from build123d import *

# Parameters (mm, degrees)
SKETCH1_R           = 36.5
BOSS_EXTRUDE1_DEPTH = 268
SKETCH2_R           = 70
SKETCH2_R_2         = 55
CUT_EXTRUDE1_DEPTH  = 36
CUT_EXTRUDE2_START  = -36
SKETCH3_R           = 70
SKETCH3_R_2         = 55
CUT_EXTRUDE2_DEPTH  = 36


with BuildPart() as part:
    # Sketch1 → Boss-Extrude1 (new body)
    with BuildSketch(Plane.XY):
        with BuildLine():
            Line((-40.165283517, 53), (-10.3, 53))
            Line((-10.3, 53), (-10.3, 65.697488536))
            ThreePointArc((-10.3, 65.697488536), (66.373170096, 4.105154246), (-2.125739686, -66.466015608))
            Line((-2.125739686, -66.466015608), (-4.128100838, -53.823604848))
            Line((-4.128100838, -53.823604848), (-32.079680877, -58.250700209))
            ThreePointArc((-32.079680877, -58.250700209), (-66.325057816, -4.820446627), (-40.165283517, 53))
        make_face()
        Circle(SKETCH1_R, mode=Mode.SUBTRACT)
    extrude(amount=BOSS_EXTRUDE1_DEPTH)

    # Sketch2 → Cut-Extrude1 (cut)
    with BuildSketch(Plane.XY.offset(268)):
        Circle(SKETCH2_R)
        Circle(SKETCH2_R_2, mode=Mode.SUBTRACT)
    extrude(amount=-CUT_EXTRUDE1_DEPTH, mode=Mode.SUBTRACT)

    # Sketch3 → Cut-Extrude2 (cut)
    with BuildSketch(Plane(origin=(0, 0, 0), x_dir=(-1, 0, 0), z_dir=(0, 0, -1)).offset(CUT_EXTRUDE2_START)):
        Circle(SKETCH3_R)
        Circle(SKETCH3_R_2, mode=Mode.SUBTRACT)
    extrude(amount=CUT_EXTRUDE2_DEPTH, mode=Mode.SUBTRACT)


solid = part.part
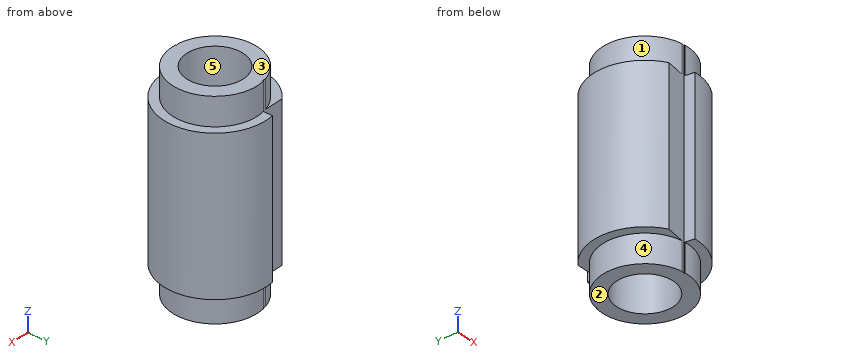
Build history of the part. All positions in model axes, mm. Face numbers are marked on the shaded views. A direction names the side the tool comes from. Round coordinates to 2 decimals unless told otherwise and drop trailing zeros. Write each loop counter-clockwise with the first axis right and the second up, starting at its lowest first coordinate (ties: lowest second). Pieces come first, ordered by that corner, then holes. Notation, with made-up numbers: M 27,4 L 43,4 A34 ccw 43,43 Z; hole C 49,25.5 d6. An arc over 180 degrees is marked long. Use CSV: the item, a comma, the result in double quotes.
1. Saw through at C-C (y = -48.5). Give the cut face in (x, z), plus the area to 3 significant figures.
Reply:
outline,"M -45.5,36 L -25.94,36 L -25.94,0 L 25.94,0 L 25.94,36 L 45.5,36 L 45.5,232 L 25.94,232 L 25.94,268 L -25.94,268 L -25.94,232 L -45.5,232 Z"
area,"21,600 mm²"
2. Saw through at D-D (y = 21.5). Give the cut face in (x, z), plus the area to 3 significant figures.
Reply:
outline,"M -62.93,36 L -50.62,36 L -50.62,0 L -29.5,0 L -29.5,268 L -50.62,268 L -50.62,232 L -62.93,232 Z; M 29.5,0 L 50.62,0 L 50.62,36 L 62.93,36 L 62.93,232 L 50.62,232 L 50.62,268 L 29.5,268 Z"
area,"16,100 mm²"
3. Saw through at B-B (z = 185.5). Give the cut face in (x, y).
Reply:
outline,"M -40.17,53 A66.5 ccw -32.08,-58.25 L -4.13,-53.82 L -2.13,-66.47 A66.5 ccw long -10.3,65.7 L -10.3,53 Z; hole C 0,0 d73"
4. Flat gauge pins, fed straight in: pin 1 (15 mm diameter, centred on x = -22, z = 135, fed in from +Y); pin 2 (3 mm diameter, centred on x = -42, z = 190, fed in from +Y); pin 3 (12 mm diameter, centred on x = 13, z = 30.5, fed in from +Y). Where does each tip first touch, or does it go through?
Reply:
pin 1,"stops at y = 53"
pin 2,"stops at y = 52.74"
pin 3,"stops at y = 65.65"
5. Two-plate mould, pull along X, no slides. Class the marked faces 3, 4 and 5: +X half, -X half, draft (parallel to the pull), parting line (faces both ways), or undercut.
Reply:
face 3,"draft"
face 4,"-X half"
face 5,"undercut"
6. Wall check: probe 1 along Y at (x, z) = (0, 119); probe 2 along X at (y, z) = (2, 159); probe 3 along X at (y, z) = (19.5, 180). Give the ranges that are in metal, low to high. Write a range as from..to.
Reply:
probe 1,"y = -66.5..-36.5, 36.5..66.5"
probe 2,"x = -66.47..-36.45, 36.45..66.47"
probe 3,"x = -63.58..-30.85, 30.85..63.58"
7. Tool access for the marked faces 1 and 2: list every direction of +Z, -Z, +X, -X, +Y, -Y with a clear straight run to the whole face (end or side of a thin tool).
Reply:
face 1,"+Z, -X"
face 2,"-Z, +X, -X, +Y, -Y"
8. Saw through at A-A (y = 0). Give the cut face in (x, z), plus the area to 3 significant figures.
Reply:
outline,"M -66.5,36 L -55,36 L -55,0 L -36.5,0 L -36.5,268 L -55,268 L -55,232 L -66.5,232 Z; M 36.5,0 L 55,0 L 55,36 L 66.5,36 L 66.5,232 L 55,232 L 55,268 L 36.5,268 Z"
area,"14,400 mm²"
